Here's how the part is built. I have some questions about the finished solid (model axes, mm). A direction names the side the tool comes from. Round coordinates to 2 decimals unless told otherwise and drop trailing zeros. Loops run counter-clockwise (first coordinate to the right, second up) from the corner with the lowest first, then second, coordinate; pieces in that order, holes last. Notation, with made-up numbers: M 73,-28 L 97,-28 A35 cw 97,11 Z; hole C 75.5,16 d2. An arc over 180 degrees is marked long. Use a Markdown table: item, result.
```python
from build123d import *

# Parameters (mm, degrees)
BASE_PLATE_DEPTH         = 12
CENTRE_HOLE_16_SKETCH_R  = 8
CENTRE_HOLE_16_DEPTH     = 12
GROOVE_SKETCH_W          = 60
GROOVE_SKETCH_H          = 8
GROOVE_8MM_DEPTH         = 6
UPRIGHT_WALL_DEPTH       = 60
PIN_LUG_SKETCH_R         = 9
PIN_LUG_DEPTH            = 7.5
HOLE_26_SKETCH_R         = 13
HOLE_26_DEPTH            = 12
RECESS_18_SKETCH_R       = 9
RECESS_18_DEPTH          = 6
SIDE_HOLE_10_SKETCH_R    = 5
SIDE_HOLE_10_DEPTH       = 13
LUG_START                = -85
LUG_PIN_HOLE_10_SKETCH_R = 5
LUG_PIN_HOLE_10_DEPTH    = 85


with BuildPart() as part:
    # Base Plate Sketch → Base Plate (new body)
    with BuildSketch(Plane(origin=(0, 0, 0), x_dir=(1, 0, 0), z_dir=(0, 1, 0))):
        with BuildLine():
            Line((30, 0), (30, -70))
            Line((30, -70), (-30, -70))
            Line((-30, -70), (-30, 0))
            ThreePointArc((-30, 0), (0, 30), (30, 0))
        make_face()
    extrude(amount=BASE_PLATE_DEPTH)

    # Centre Hole Ø16 Sketch → Centre Hole Ø16 (cut)
    with BuildSketch(Plane(origin=(0, 12, 0), x_dir=(1, 0, 0), z_dir=(0, 1, 0))):
        with Locations(Location((0, 0, 0), (0, 0, 270))):
            Circle(CENTRE_HOLE_16_SKETCH_R)
    extrude(amount=-CENTRE_HOLE_16_DEPTH, mode=Mode.SUBTRACT)

    # Groove Sketch → Groove 8mm (cut)
    with BuildSketch(Plane(origin=(0, 12, 0), x_dir=(1, 0, 0), z_dir=(0, 1, 0))):
        with Locations((0, -66)):
            Rectangle(GROOVE_SKETCH_W, GROOVE_SKETCH_H)
    extrude(amount=-GROOVE_8MM_DEPTH, mode=Mode.SUBTRACT)

    # Upright Wall Sketch → Upright Wall (add)
    with BuildSketch(Plane(origin=(30, 0, 0), x_dir=(0, 0, -1), z_dir=(1, 0, 0))):
        Polygon((-62, 12), (-18, 12), (-18, 25), (-30, 25), (-62, 25), align=None)
    extrude(amount=-UPRIGHT_WALL_DEPTH)

    # Pin Lug Sketch → Pin Lug (add)
    with BuildSketch(Plane(origin=(30, 0, 0), x_dir=(0, 0, -1), z_dir=(1, 0, 0))):
        with BuildLine():
            Line((-60, 25), (-30, 25))
            Line((-30, 25), (-30, 65))
            ThreePointArc((-30, 65), (-60, 82.320508076), (-60, 47.679491924))
            Line((-60, 47.679491924), (-60, 25))
        make_face()
        with Locations((-50, 65)):
            Circle(PIN_LUG_SKETCH_R, mode=Mode.SUBTRACT)
    pin_lug = extrude(amount=-PIN_LUG_DEPTH)

    # Pin Lug Mirror: Pin Lug across plane
    add(pin_lug.mirror(Plane(origin=(0, 0, 0), x_dir=(0, 0, 1), z_dir=(1, 0, 0))))

    # Hole Ø26 Sketch → Hole Ø26 (cut)
    with BuildSketch(Plane(origin=(0, 0, 18), x_dir=(-1, 0, 0), z_dir=(0, 0, -1))):
        with Locations((0, 25)):
            Circle(HOLE_26_SKETCH_R)
    extrude(amount=-HOLE_26_DEPTH, mode=Mode.SUBTRACT)

    # Recess Ø18 Sketch → Recess Ø18 (cut)
    with BuildSketch(Plane(origin=(0, 25, 0), x_dir=(1, 0, 0), z_dir=(0, 1, 0))):
        with Locations(Location((0, -46, 0), (0, 0, 270))):
            Circle(RECESS_18_SKETCH_R)
    extrude(amount=-RECESS_18_DEPTH, mode=Mode.SUBTRACT)

    # Side Hole Ø10 Sketch → Side Hole Ø10 (cut)
    with BuildSketch(Plane(origin=(30, 0, 0), x_dir=(0, 0, -1), z_dir=(1, 0, 0))):
        with Locations((-45, 12)):
            Circle(SIDE_HOLE_10_SKETCH_R)
    extrude(amount=-SIDE_HOLE_10_DEPTH, mode=Mode.SUBTRACT)

    # Lug Pin Hole Ø10 Sketch → Lug Pin Hole Ø10 (cut)
    with BuildSketch(Plane.ZY.offset(30).offset(LUG_START)):
        with Locations(Location((45, 12, 0), (0, 0, 180))):
            Circle(LUG_PIN_HOLE_10_SKETCH_R)
    extrude(amount=LUG_PIN_HOLE_10_DEPTH, mode=Mode.SUBTRACT)


solid = part.part
```
Q1. Imagine slicing it at C-C, the plane y = 67.5. Please give me the cut outline in (x, z), then the cut area to 3 significant figures.
Return value:
| item | result |
|---|---|
| outline | M -30,30.16 L -22.5,30.16 L -22.5,41.35 L -30,41.35 Z; M -30,58.65 L -22.5,58.65 L -22.5,69.84 L -30,69.84 Z; M 22.5,30.16 L 30,30.16 L 30,41.35 L 22.5,41.35 Z; M 22.5,58.65 L 30,58.65 L 30,69.84 L 22.5,69.84 Z |
| area | 336 mm^2 |
Q2. Imagine slicing it at D-D, the plane z = 5. Please give me the cut outline in (x, y) (3 decimals).
Return value:
| item | result |
|---|---|
| outline | M -30,0 L -6.245,0 L -6.245,12 L -30,12 Z; M 6.245,0 L 30,0 L 30,12 L 6.245,12 Z |
Q3. Imagine slicing it at B-B, the plane z = 43.5. Please give me the cut outline in (x, y).
Return value:
| item | result |
|---|---|
| outline | M -30,0 L 30,0 L 30,7.23 L -30,7.23 Z; M -30,16.77 L 30,16.77 L 30,58.78 L 22.5,58.78 L 22.5,25 L 8.65,25 L 8.65,19 L -8.65,19 L -8.65,25 L -22.5,25 L -22.5,58.78 L -30,58.78 Z; M -30,71.22 L -22.5,71.22 L -22.5,83.91 L -30,83.91 Z; M 22.5,71.22 L 30,71.22 L 30,83.91 L 22.5,83.91 Z |
Q4. Will these pins go through, and if not, where does the flat tip stop? P1, Ø2, axis at x = 28, y = 40, coming from the +Z side; P2, Ø2, axis at x = -27.5, y = 54, coming from the -Z side; P3, Ø10.5, axis at x = -13.5, y = 17, coming from the -Z side; P4, Ø2, axis at y = 27, z = 27, coming from the +X side.
Return value:
| item | result |
|---|---|
| P1 | stops at z = 60 |
| P2 | stops at z = 30 |
| P3 | stops at z = -27.54 |
| P4 | passes through |
Q5. For faces 1 (the cylindrical face through (0, 12, 24)), 2 (the flat face through (0, 6, 66)), 3 (the flat face through (19, 18, 18)), which set-ups out of +Z, -Z, +X, -X, +Y, -Y let a thin tool reach every point of the face, with its end or its side?
Return value:
| item | result |
|---|---|
| face 1 | -Z, +Y |
| face 2 | +Z, +X, -X |
| face 3 | -Z, +X, -X, +Y |
Q6. Imagine slicing it at A-A, the plane x = 3. Please give me the cut outline in (y, z).
Return value:
| item | result |
|---|---|
| outline | M 0,-29.85 L 12,-29.85 L 12,-7.42 L 0,-7.42 Z; M 0,7.42 L 12,7.42 L 12,18 L 12.35,18 L 12.35,30 L 25,30 L 25,37.51 L 19,37.51 L 19,54.49 L 25,54.49 L 25,62 L 6,62 L 6,70 L 0,70 Z; hole C 12,45 d10 |
Q7. We'd pull the mould along X, two halves only. Please class faces 4 (the cylindrical face through (0, 22, 37)), 5 (the flat face through (0, 16, 62)), 6 (the cylindrical face through (-0.66, 5.916, -29.993)): pulls with the +X half, pulls with the -X half, needs draft (parallel to the pull), parting line crosses it, or undercut.
Return value:
| item | result |
|---|---|
| face 4 | undercut |
| face 5 | needs draft |
| face 6 | parting line crosses it |
Q8. I need wall thicknesses on line 1 (Y direction, x = 24, z = 46.5); line 2 (X direction, y = 29, z = 43); line 3 (Y direction, x = 13.5, z = -0.5). Which ranges of each line are inside material? Lowest first, please. Write a range as from..to.
Return value:
| item | result |
|---|---|
| line 1 | y = 0..7.23, 16.77..56.71, 73.29..84.69 |
| line 2 | x = -30..-22.5, 22.5..30 |
| line 3 | y = 0..12 |
